from build123d import *

# Parameters (mm, degrees)
BOSS_EXTRUDE1_DEPTH = 1.5
SKETCH2_R           = 2.25
CUT_EXTRUDE1_DEPTH  = 3


with BuildPart() as part:
    # Sketch1 → Boss-Extrude1 (new, symmetric)
    with BuildSketch(Plane.XY):
        Polygon((-646.5, 109.2), (-561.5, 109.2), (-561.5, 121.7), (-566.5, 126.7), (-641.5, 126.7), (-646.5, 121.7), align=None)
    extrude(amount=BOSS_EXTRUDE1_DEPTH, both=True)

    # Sketch2 → Cut-Extrude1 (cut)
    with BuildSketch(Plane.XY.offset(1.5)):
        with Locations((-636.5, 119.2)):
            Circle(SKETCH2_R)
        with Locations((-571.5, 119.2)):
            Circle(SKETCH2_R)
    extrude(amount=-CUT_EXTRUDE1_DEPTH, mode=Mode.SUBTRACT)


solid = part.part
The listing builds one solid part. Answer for the finished solid, in the listing's coordinates (mm). Round coordinates to 2 decimals unless told otherwise and drop trailing zeros. Order: outer loops, then holes, each group sorted by start corner. A loop starts at its lowest first (then second) coordinate and runs counter-clockwise, first axis right, second up. Notation, with made-up numbers: (72.25, -9) -> (126.25, -9) arc R22 cw to (126.25, 18) -> close; hole circle Ø2 at (80.25, -14.75). An arc over 180 degrees is marked (long way). Write each question's results on one line, items separated by ' | '. Start each with the question number.
Q1. Straight lines are drawn through the part: probe 1 along X at (y, z) = (119, -0.4); probe 2 along X at (y, z) = (121, -0.6); probe 3 along Y at (x, z) = (-571.5, 0). For each, find the intervals that lie inside material, in ascending order. Write a range as from..to.
Q2. Find section D-D (y = 125.75). Determine the outline of the cut face in (x, z), then the cut area to 3 significant figures.
Q3. Find section C-C (y = 119.2). Determine the outline of the cut face in (x, z).
Q4. Find section B-B (z = -1). Determine the outline of the cut face in (x, y), then the cut area to 3 significant figures.
Q5. Find section A-A (x = -571.5). Determine the outline of the cut face in (y, z), then the cut area to 3 significant figures.
Q6. The mould has two halves that part along Y. Classify faces 1 (the flat face through (-646.5, 116, 0)), 2 (the flat face through (-605, 109.2, 0)), 3 (the cylindrical face through (-634.354, 119.876, 0.021)), 4 (the flat face through (-603, 126.7, 0)): pulls with the +Y half, pulls with the -Y half, needs draft (parallel to the pull), parting line crosses it, or undercut.
Q7. This flat-tipped pin is pushed along its axis until it touches: pin 1 (6 mm diameter, centred on x = -636.5, y = 119.2, fed in from +Z). Where does it stop, or does it pass through?
Worked answers:
1) probe 1: x = -646.5..-638.74, -634.26..-573.74, -569.26..-561.5 | probe 2: x = -646.5..-637.85, -635.15..-572.85, -570.15..-561.5 | probe 3: y = 109.2..116.95, 121.45..126.7
2) outline: (-642.45, -1.5) -> (-565.55, -1.5) -> (-565.55, 1.5) -> (-642.45, 1.5) -> close | area: 231 mm2
3) outline: (-646.5, -1.5) -> (-638.75, -1.5) -> (-638.75, 1.5) -> (-646.5, 1.5) -> close; (-634.25, -1.5) -> (-573.75, -1.5) -> (-573.75, 1.5) -> (-634.25, 1.5) -> close; (-569.25, -1.5) -> (-561.5, -1.5) -> (-561.5, 1.5) -> (-569.25, 1.5) -> close
4) outline: (-646.5, 109.2) -> (-561.5, 109.2) -> (-561.5, 121.7) -> (-566.5, 126.7) -> (-641.5, 126.7) -> (-646.5, 121.7) -> close; hole circle Ø4.5 at (-636.5, 119.2); hole circle Ø4.5 at (-571.5, 119.2) | area: 1,430 mm2
5) outline: (109.2, -1.5) -> (116.95, -1.5) -> (116.95, 1.5) -> (109.2, 1.5) -> close; (121.45, -1.5) -> (126.7, -1.5) -> (126.7, 1.5) -> (121.45, 1.5) -> close | area: 39.0 mm2
6) face 1: needs draft | face 2: pulls with the -Y half | face 3: undercut | face 4: pulls with the +Y half
7) pin 1: stops at z = 1.5
